Source: CAD feature listing. Evaluate the final solid. Frame: model axes, mm. Give positions to 0.01 mm unless a question says otherwise; leave off trailing zeros. Order: outer loops, then holes, each group sorted by start corner. A loop starts at its lowest first (then second) coordinate and runs counter-clockwise, first axis right, second up. Notation, with made-up numbers: (76, -25) - (135, -25) arc R29 ccw to (135, 9) - close; hole circle Ø10 at (-7, -28). An arc over 180 degrees is marked (long way). Write each question's results on one line, items separated by ' | '. Start each with the question number.
Item 1: Section A-A on y = 1.5. Output: boundary loops of the cut face in (x, z).
Item 2: Line query: line 1 along X through (y, z) = (-1.75, 0.65); line 2 along X through (y, z) = (-0.5, 0.65); line 3 along Y through (x, z) = (15, 0.65). Output: solid intervals per line, ascending.
Item 3: Section C-C on z = 2.95. Output: boundary loops of the cut face in (x, y).
Item 4: Section B-B on x = 10.25. Output: boundary loops of the cut face in (y, z).
Item 5: Contact query for flat-ended pins moving along their axis: pin 1 Ø2 at (y, z) = (3.5, 0.5) entering from -X; pin 2 Ø2 at (x, z) = (22.5, 0.5) entering from -Y; pin 3 Ø2 at (x, z) = (14.5, 0.5) entering from +Y. Output: stop coordinate, or through.
Item 6: Section D-D on y = -0.5. Output: boundary loops of the cut face in (x, z), and give its area (3 significant figures).
Item 7: Mould query, pull axis Y, two halves, no side actions, for faces 1 (the cylindrical face through (29.633, 1.121, 1.726)), 2 (the cylindrical face through (3.793, 0.169, 1.726)), 3 (the cylindrical face through (2.02, 0.13, 1.73)), 4 (the flat face through (17, 0, 3.5)). Classes: released by +Y, released by -Y, zero draft, split by the parting line, or undercut.
```python
from build123d import *

# Parameters (mm, degrees)
SKETCH1_R           = 3.674588618
BOSS_EXTRUDE1_DEPTH = 3.5


with BuildPart() as part:
    # Sketch1 → Boss-Extrude1 (new body)
    with BuildSketch(Plane.XY):
        with BuildLine():
            Line((26.125402815, 5.46233555), (7.464079644, 5.452693539))
            ThreePointArc((7.464079644, 5.452693539), (2.01909867, 0.007712565), (7.464079644, -5.43726841))
            Line((7.464079644, -5.43726841), (7.46970589, -5.437265503))
            Line((7.46970589, -5.437265503), (26.128216151, -5.427625672))
            ThreePointArc((26.128216151, -5.427625672), (31.573196944, 0.01876197), (26.125402815, 5.46233555))
        make_face()
        with Locations((7.464079644, 0.007712565)):
            Circle(SKETCH1_R, mode=Mode.SUBTRACT)
        with Locations((26.128216151, 0.017355302)):
            Circle(SKETCH1_R, mode=Mode.SUBTRACT)
    extrude(amount=BOSS_EXTRUDE1_DEPTH)


solid = part.part
```
Evaluation:
1) outline: (2.23, 0) - (4.11, 0) - (4.11, 3.5) - (2.23, 3.5) - close; (10.82, 0) - (22.77, 0) - (22.77, 3.5) - (10.82, 3.5) - close; (29.49, 0) - (31.37, 0) - (31.37, 3.5) - (29.49, 3.5) - close
2) line 1: x = 2.31 to 4.24, 10.69 to 22.91, 29.35 to 31.28 | line 2: x = 2.04 to 3.82, 11.1 to 22.49, 29.77 to 31.55 | line 3: y = -5.43 to 5.46
3) outline: (7.46, -5.44) - (26.13, -5.43) arc R5.44 ccw to (26.13, 5.46) - (7.46, 5.45) arc R5.44 ccw to start; hole circle Ø7.35 at (7.46, 0.01); hole circle Ø7.35 at (26.13, 0.02)
4) outline: (-5.44, 0) - (-2.39, 0) - (-2.39, 3.5) - (-5.44, 3.5) - close; (2.4, 0) - (5.45, 0) - (5.45, 3.5) - (2.4, 3.5) - close
5) pin 1: stops at x = 2.62 | pin 2: stops at y = -5.43 | pin 3: stops at y = 5.46
6) outline: (2.04, 0) - (3.82, 0) - (3.82, 3.5) - (2.04, 3.5) - close; (11.1, 0) - (22.49, 0) - (22.49, 3.5) - (11.1, 3.5) - close; (29.77, 0) - (31.55, 0) - (31.55, 3.5) - (29.77, 3.5) - close | area: 52.3 mm^2
7) face 1: undercut | face 2: undercut | face 3: split by the parting line | face 4: zero draft
